```python
from build123d import *

# Parameters (mm, degrees)
SKETCH_1_W          = 80
SKETCH_1_H          = 60
EXTRUDE_1_DEPTH     = 6
SKETCH_2_W          = 12
SKETCH_2_H          = 60
CUT_EXTRUDE_1_DEPTH = 1.5
CUT_EXTRUDE_2_REACH = 53.42
SKETCH_3_W          = 55
SKETCH_3_H          = 17
FILLET_1_R          = 10


with BuildPart() as part:
    # 草图1 → 凸台-拉伸1 (new, symmetric)
    with BuildSketch(Plane.XY):
        Rectangle(SKETCH_1_W, SKETCH_1_H)
    extrude(amount=EXTRUDE_1_DEPTH, both=True)

    # 草图2 → 切除-拉伸1 (cut)
    with BuildSketch(Plane.XY.offset(-6)):
        with Locations((34, 0)):
            Rectangle(SKETCH_2_W, SKETCH_2_H)
    extrude(amount=CUT_EXTRUDE_1_DEPTH, mode=Mode.SUBTRACT)

    # 草图3 → 切除-拉伸2 (cut, up to next)
    with BuildSketch(Plane(origin=(0, 0, -6), x_dir=(-1, 0, 0), z_dir=(0, 0, -1)), mode=Mode.PRIVATE) as cut_extrude_2_sk1:
        with Locations((12.5, -21.5)):
            Rectangle(SKETCH_3_W, SKETCH_3_H)
    cut_extrude_2_tool1 = extrude(cut_extrude_2_sk1.sketch, amount=-CUT_EXTRUDE_2_REACH, mode=Mode.PRIVATE) & part.part
    add(cut_extrude_2_tool1.solids().sort_by_distance((-12.5, -21.5, -6))[0], mode=Mode.SUBTRACT)

    # 圆角1
    fillet_1_edges = [part.edges().sort_by_distance(p)[0] for p in [
        (15, -13, 0),
    ]]
    fillet(fillet_1_edges, radius=FILLET_1_R)


solid = part.part
```
The model under review builds one solid part; all positions refer to its coordinate system, in mm. A direction names the side the tool comes from. Round coordinates to 2 decimals unless told otherwise and drop trailing zeros. Order: outer loops, then holes, each group sorted by start corner. A loop starts at its lowest first (then second) coordinate and runs counter-clockwise, first axis right, second up.
(1) For P1, Ø3, axis at x = 10.5, z = 4.5, coming from the -Y side; P2, Ø6, axis at x = 4.5, z = -1, coming from the -Y side; P3, Ø1.6, axis at y = -12.5, z = -5.5, coming from the +X side, all flat-tipped, find the tip position at first contact; note any pin that passes through.
Working result:
P1: stops at y = -15.86
P2: stops at y = -13.32
P3: stops at x = 28
(2) Tool access review of faces 1 (the face through (-40, 8, 0)), 2 (the face through (15, -27, 0)), 3 (the face through (34, 0, -4.5)): name each direction out of +Z, -Z, +X, -X, +Y, -Y from which nothing blocks a thin tool from reaching the whole face with its end or side.
Working result:
face 1: +Z, -Z, -X, +Y, -Y
face 2: +Z, -Z, -X, -Y
face 3: -Z, +X, +Y, -Y
(3) Wall thickness on L1, parallel to Y at x = -29.5, z = 4.5; L2, parallel to X at y = -23, z = -4; L3, parallel to X at y = 25, z = -5: over which ranges is each line inside the solid? List them lowest first.
Working result:
L1: y = -13 to 30
L2: x = 15 to 40
L3: x = -40 to 28
(4) Take a section at A-A, the plane z = 4.5. State the section outline as (x, y) points.
Working result:
outline: (-40, -13) - (5, -13) arc R10 cw to (15, -23) - (15, -30) - (40, -30) - (40, 30) - (-40, 30) - close
(5) Take a section at B-B, the plane y = -0.5. State the section outline as (x, z) points, plus the area to 3 significant figures.
Working result:
outline: (-40, -6) - (28, -6) - (28, -4.5) - (40, -4.5) - (40, 6) - (-40, 6) - close
area: 942 mm2
(6) Take a section at C-C, the plane x = -16.5. State the section outline as (y, z) points.
Working result:
outline: (-13, -6) - (30, -6) - (30, 6) - (-13, 6) - close
(7) Take a section at D-D, the plane y = -15.5. State the section outline as (x, z) points.
Working result:
outline: (11.61, -6) - (28, -6) - (28, -4.5) - (40, -4.5) - (40, 6) - (11.61, 6) - close
